Could you check a few things on this drawing? It's one solid part, dimensions in mm from its lowest x, y, z. A direction names the side the tool comes from. Round coordinates to 2 decimals unless told otherwise and drop trailing zeros. Order: outer loops, then holes, each group sorted by start corner. A loop starts at its lowest first (then second) coordinate and runs counter-clockwise, first axis right, second up.
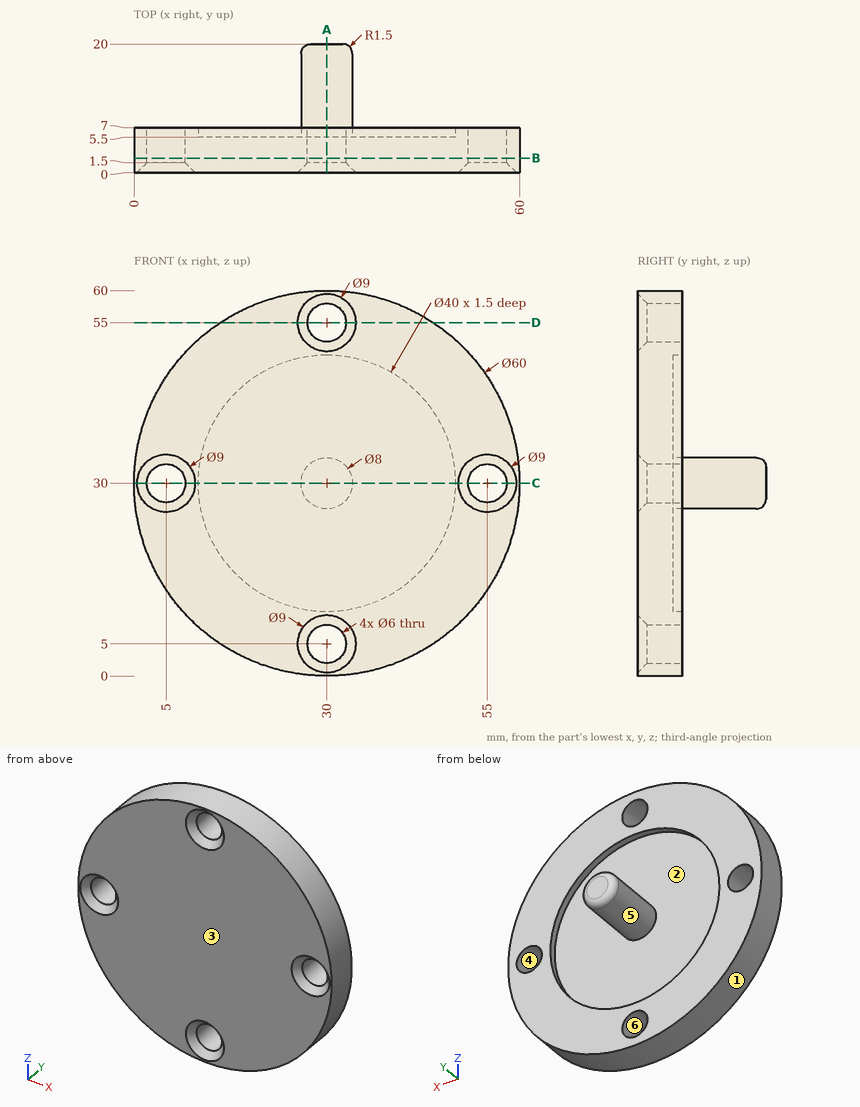
(1) If we mould it in two halves opening along Z, with no side actions, what happens to the marked faces 1, 2, 3 and 4? For each: pulls with the +Z half, pulls with the -Z half, needs draft (parallel to the pull), parting line crosses it, or undercut.
(2) I'm going to push flat-ended pins straight in: pin 1 Ø3 at (x, y) = (43.5, 9.5) entering from +Z; pin 2 Ø8 at (x, y) = (49, 2) entering from +Z; pin 3 Ø5 at (x, z) = (20, 17) entering from +Y; pin 4 Ø20 at (x, z) = (40, 26) entering from +Y. Where does each tip first touch, or does it pass through?
(3) Please list where these lines run through material, in increasing order: probe 1 along X at (y, z) = (3.35, 30); probe 2 along Z at (x, y) = (31, 4); probe 3 along Y at (x, z) = (42.5, 54).
(4) I want a section at C-C, the plane z = 30. List the corners of the cut face in (x, y) for me.
(5) I want a section at A-A, the plane x = 30. List the corners of the cut face in (y, z) for me.
(6) I want a section at D-D, the plane z = 55. List the corners of the cut face in (x, y) for me.
(7) I want a section at B-B, the plane y = 2.25. List the corners of the cut face in (x, z) for me, plus the area to 3 significant figures.
(8) On a 3-axis mill with a long thin cutter (end or side, diameter ignored), from which of +Z, -Z, +X, -X, +Y, -Y can I reach the whole of each face in a straight line? I mean the marked faces 5 and 6. Say none if no direction works.
Ans:
1. face 1: parting line crosses it
1. face 2: undercut
1. face 3: needs draft
1. face 4: undercut
2. pin 1: passes through
2. pin 2: stops at z = 55.98
2. pin 3: stops at y = 5.5
2. pin 4: stops at y = 20
3. probe 1: x = 0 to 2, 8 to 52, 58 to 60
3. probe 2: z = 0.02 to 2.17, 7.83 to 52.17, 57.83 to 59.98
3. probe 3: y = 0 to 7
4. outline: (0, 0) - (0.5, 0) - (2, 1.5) - (2, 7) - (0, 7) - close; (8, 1.5) - (9.5, 0) - (50.5, 0) - (52, 1.5) - (52, 7) - (50, 7) - (50, 5.5) - (34, 5.5) - (34, 18.5) arc R1.5 ccw to (32.5, 20) - (27.5, 20) arc R1.5 ccw to (26, 18.5) - (26, 5.5) - (10, 5.5) - (10, 7) - (8, 7) - close; (58, 1.5) - (59.5, 0) - (60, 0) - (60, 7) - (58, 7) - close
5. outline: (0, 0) - (7, 0) - (7, 2) - (1.5, 2) - (0, 0.5) - close; (0, 9.5) - (1.5, 8) - (7, 8) - (7, 10) - (5.5, 10) - (5.5, 26) - (18.5, 26) arc R1.5 ccw to (20, 27.5) - (20, 32.5) arc R1.5 ccw to (18.5, 34) - (5.5, 34) - (5.5, 50) - (7, 50) - (7, 52) - (1.5, 52) - (0, 50.5) - close; (0, 59.5) - (1.5, 58) - (7, 58) - (7, 60) - (0, 60) - close
6. outline: (13.42, 0) - (25.5, 0) - (27, 1.5) - (27, 7) - (13.42, 7) - close; (33, 1.5) - (34.5, 0) - (46.58, 0) - (46.58, 7) - (33, 7) - close
7. outline: circle Ø60 at (30, 30); hole circle Ø6 at (5, 30); hole circle Ø6 at (30, 5); hole circle Ø6 at (30, 55); hole circle Ø6 at (55, 30)
7. area: 2,710 mm2
8. face 5: +Y
8. face 6: +Y, -Y
